Check sheet for the drawn part. Datum: minimum x, y, z corner. Units: mm. A direction names the side the tool comes from. Coordinates: 2 decimals unless noted, no trailing zeros. Order: outer loops, then holes, each group sorted by start corner. A loop starts at its lowest first (then second) coordinate and runs counter-clockwise, first axis right, second up. Notation, with made-up numbers: (11, 34.5) - (58, 34.5) arc R5 ccw to (58, 41.5) - close; hole circle Ø3 at (36.5, 9.25). An arc over 180 degrees is marked (long way). Answer as CSV lines item,"result". Start each with the question number.
1. Go/stop test with flat-tipped pins: pin 1 (22 mm diameter, centred on x = 65, z = 31, fed in from -Y); pin 2 (3 mm diameter, centred on y = 66, z = 58, fed in from -X); pin 3 (16 mm diameter, centred on y = 92, z = 12, fed in from -X); pin 4 (10 mm diameter, centred on y = 5.5, z = 41.5, fed in from -X). Record where each tip stops, or that it passes through.
2. Section check B-B (x = 89). Record the cut outline in (y, z).
3. Section check A-A (y = 97.5). Record the cut outline in (x, z), and give its area (3 significant figures).
4. Section check C-C (z = 40). Record the cut outline in (x, y), and give its area (3 significant figures).
5. Section check D-D (y = 60). Record the cut outline in (x, z), and give its area (3 significant figures).
6. Mould release check, pull along Z, two halves, no side actions. Record for the marked faces 1, 2 and 3: pulls with the +Z half, pulls with the -Z half, needs draft (parallel to the pull), parting line crosses it, or undercut.
7. Material ranges on L1, parallel to Y at x = 74, z = 60; L2, parallel to Y at x = 75.5, z = 38.5; L3, parallel to Y at x = 83, z = 60, recorded low to high. Write a range as [from, to].
8. Set-up check for the marked faces 4, 5, 6 and 7: record each of +Z, -Z, +X, -X, +Y, -Y from which the full face is reachable in a straight line by a thin tool's end or side.
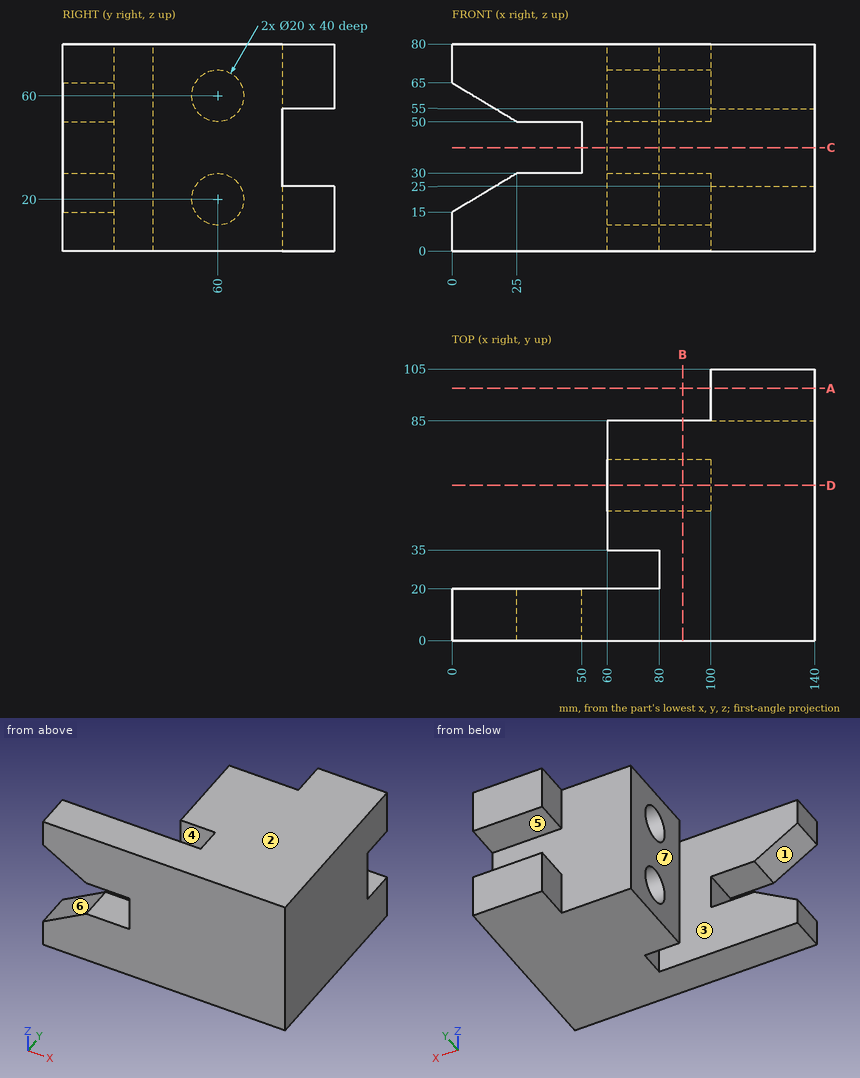
Evaluation:
1,pin 1,"stops at y = 0"
1,pin 2,"stops at x = 100"
1,pin 3,"stops at x = 60"
1,pin 4,"stops at x = 50"
2,outline,"(0, 0) - (85, 0) - (85, 80) - (0, 80) - close; hole circle Ø20 at (60, 20); hole circle Ø20 at (60, 60)"
3,outline,"(100, 0) - (140, 0) - (140, 25) - (100, 25) - close; (100, 55) - (140, 55) - (140, 80) - (100, 80) - close"
3,area,"2,000 mm²"
4,outline,"(50, 0) - (140, 0) - (140, 85) - (60, 85) - (60, 35) - (80, 35) - (80, 20) - (50, 20) - close"
4,area,"6,700 mm²"
5,outline,"(60, 0) - (140, 0) - (140, 80) - (60, 80) - (60, 70) - (100, 70) - (100, 50) - (60, 50) - (60, 30) - (100, 30) - (100, 10) - (60, 10) - close"
5,area,"4,800 mm²"
6,face 1,"undercut"
6,face 2,"pulls with the +Z half"
6,face 3,"needs draft"
7,L1,"y = [0, 20], [35, 50], [70, 85]"
7,L2,"y = [0, 20], [35, 85]"
7,L3,"y = [0, 50], [70, 85]"
8,face 4,"+Z, -Z, -X"
8,face 5,"+X, -X, +Y"
8,face 6,"-X, +Y, -Y"
8,face 7,"+Z, -Z, -X, +Y"
